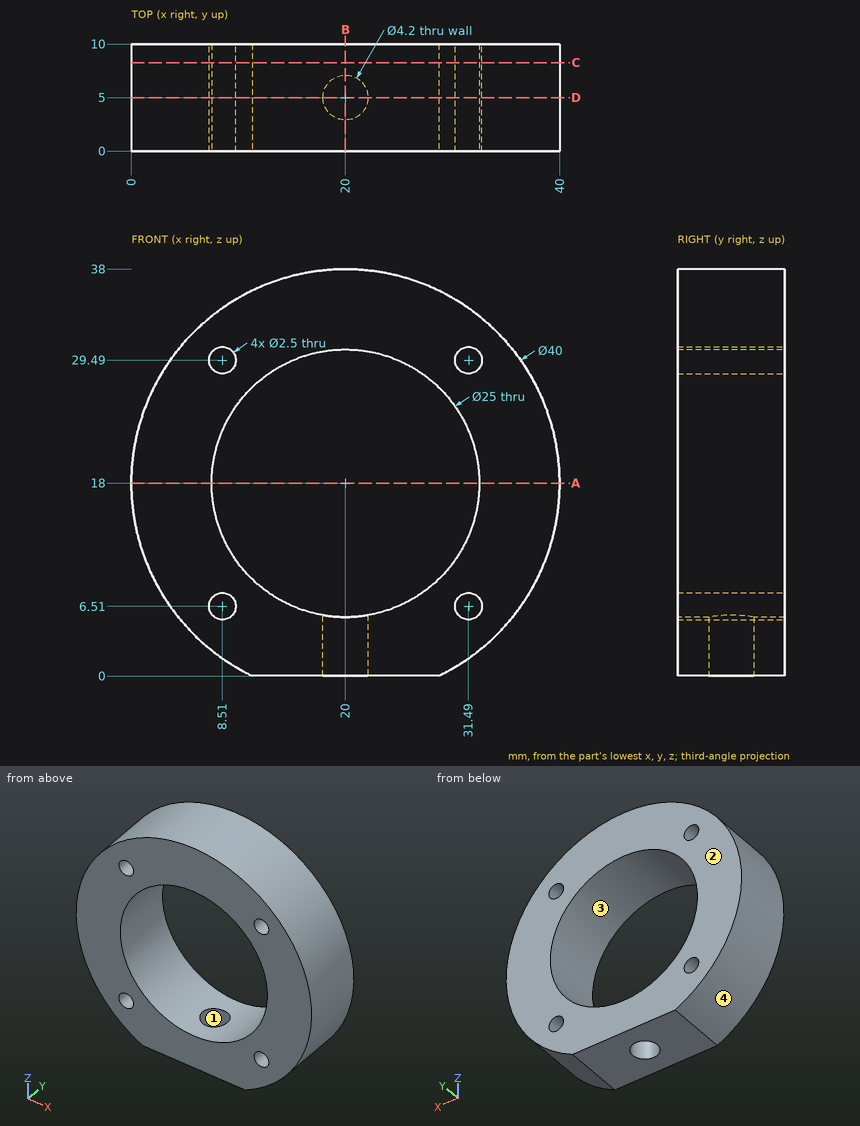
Can you work these out from the drawing? Everything is in mm from the part's minimum corner. Coordinates: 2 decimals unless noted, no trailing zeros. Loops run counter-clockwise (first coordinate to the right, second up) from the corner with the lowest first, then second, coordinate; pieces in that order, holes last.
1) Imagine slicing it at D-D on y = 5. List the corners of the cut face in (x, z) for me.
2) Imagine slicing it at B-B on x = 20. List the corners of the cut face in (y, z) for me, plus the area to 3 significant figures.
3) Thinking about a two-plate mould opening in X: for the marked faces 1, 2, 3 and 4, which applies, pulls with the +X half, pulls with the -X half, needs draft (parallel to the pull), parting line crosses it, or undercut?
4) Imagine slicing it at C-C on y = 8.25. List the corners of the cut face in (x, z) for me.
5) Imagine slicing it at A-A on z = 18. List the corners of the cut face in (x, y) for me, plus the area to 3 significant figures.
6) For pin 1 (2 mm diameter, centred on y = 8.5, z = 21.5, fed in from +X); pin 2 (4 mm diameter, centred on x = 8.51, z = 29.49, fed in from -Y); pin 3 (1 mm diameter, centred on x = 35, y = 2, fed in from -Z) (1 decimal); pin 4 (3 mm diameter, centred on x = 9.5, y = 3.5, fed in from +Z), each with a flat end and sliding along its axis, tell me the tip position at first contact or that it passes through.
7) I need wall thicknesses on probe 1 along Z at (x, y) = (9, 1) (1 decimal); probe 2 along X at (y, z) = (9.5, 23) (1 decimal); probe 3 along X at (y, z) = (7.75, 11.5) (1 decimal). Which ranges of each line are inside material? Lowest first, please.
Completed:
1. outline: (11.28, 0) - (17.9, 0) - (17.9, 5.68) arc R12.5 cw (long way) to (22.1, 5.68) - (22.1, 0) - (28.72, 0) arc R20 ccw (long way) to start; hole circle Ø2.5 at (8.51, 6.51); hole circle Ø2.5 at (8.51, 29.49); hole circle Ø2.5 at (31.49, 6.51); hole circle Ø2.5 at (31.49, 29.49)
2. outline: (0, 0) - (2.9, 0) - (2.9, 5.5) - (0, 5.5) - close; (0, 30.5) - (10, 30.5) - (10, 38) - (0, 38) - close; (7.1, 0) - (10, 0) - (10, 5.5) - (7.1, 5.5) - close
2. area: 107 mm2
3. face 1: undercut
3. face 2: needs draft
3. face 3: undercut
3. face 4: parting line crosses it
4. outline: (11.28, 0) - (28.72, 0) arc R20 ccw (long way) to start; hole circle Ø2.5 at (8.51, 6.51); hole circle Ø2.5 at (8.51, 29.49); hole circle Ø25 at (20, 18); hole circle Ø2.5 at (31.49, 6.51); hole circle Ø2.5 at (31.49, 29.49)
5. outline: (0, 0) - (7.5, 0) - (7.5, 10) - (0, 10) - close; (32.5, 0) - (40, 0) - (40, 10) - (32.5, 10) - close
5. area: 150 mm2
6. pin 1: stops at x = 39.84
6. pin 2: stops at y = 0
6. pin 3: stops at z = 4.2
6. pin 4: stops at z = 35.86
7. probe 1: z = 1.3 to 5.4, 7.7 to 12.1, 23.9 to 28.3, 30.6 to 34.7
7. probe 2: x = 0.6 to 8.5, 31.5 to 39.4
7. probe 3: x = 1.1 to 9.3, 30.7 to 38.9
